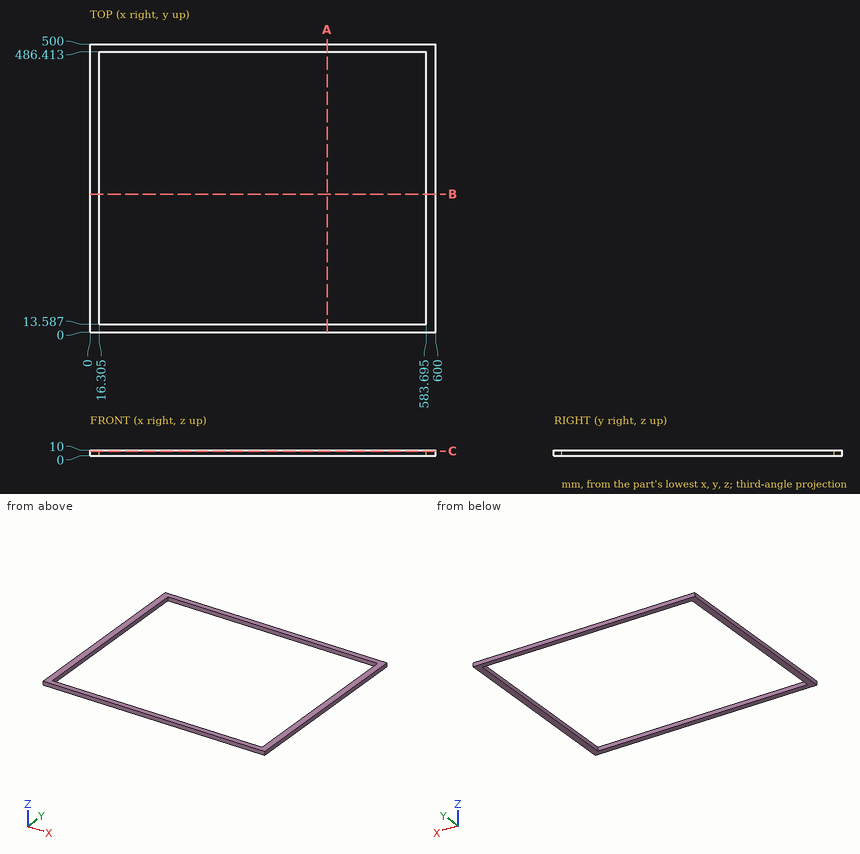
Design review of the part shown in the three views and the two pictorial views. Dimensions are in mm from the part's minimum x, y and z. Coordinates: 2 decimals unless noted, no trailing zeros. Order: outer loops, then holes, each group sorted by start corner. A loop starts at its lowest first (then second) coordinate and runs counter-clockwise, first axis right, second up. Notation, with made-up numbers: (-25.75, 78) - (27.25, 78) arc R16 ccw to (27.25, 98) - close; hole circle Ø11 at (-15.75, 16). An arc over 180 degrees is marked (long way). One line per question, with ' | ' between items.
Q1. Consider section C-C, the plane z = 8.25. Give the boundary of the cut face in (x, y) (1 decimal).
Answer key:
outline: (0, 0) - (600, 0) - (600, 500) - (0, 500) - close; hole (16.3, 13.6) - (583.7, 13.6) - (583.7, 486.4) - (16.3, 486.4) - close
Q2. Consider section A-A, the plane x = 411.5. Give the boundary of the cut face in (y, z), then the cut area to 3 significant figures.
Answer key:
outline: (0, 0) - (13.59, 0) - (13.59, 10) - (0, 10) - close; (486.41, 0) - (500, 0) - (500, 10) - (486.41, 10) - close | area: 272 mm2
Q3. To check wall thickness, follow line 1 along Y through (x, z) = (565.5, 8.5); line 2 along X through (y, z) = (51, 9.25) (1 decimal). State the ranges of each line that lie inside material, in increasing order.
Answer key:
line 1: y = 0 to 13.59, 486.41 to 500 | line 2: x = 0 to 16.3, 583.7 to 600
Q4. Consider section B-B, the plane y = 239.5. Give the boundary of the cut face in (x, z) (1 decimal), then the cut area to 3 significant figures.
Answer key:
outline: (0, 0) - (16.3, 0) - (16.3, 10) - (0, 10) - close; (583.7, 0) - (600, 0) - (600, 10) - (583.7, 10) - close | area: 326 mm2
